from build123d import *

# Parameters (mm, degrees)
SKETCH1_W                                    = 40
SKETCH1_H                                    = 60
BOSS_EXTRUDE1_DEPTH                          = 24
SKETCH4_W                                    = 38
SKETCH4_H                                    = 18
CUT_EXTRUDE2_DEPTH                           = 83
SKETCH5_W                                    = 4
SKETCH5_H                                    = 60
BOSS_EXTRUDE2_DEPTH                          = 5
SKETCH6_W                                    = 4
SKETCH6_H                                    = 11
BOSS_EXTRUDE3_DEPTH                          = 5
SKETCH7_W                                    = 40
SKETCH7_H                                    = 6
BOSS_EXTRUDE4_DEPTH                          = 18
CBORE_FOR_M5_HEXAGON_SOCKET_HEAD_CAP_2_COUNT = 2
CBORE_FOR_M5_HEXAGON_SOCKET_HEAD_CAP_2_PITCH = 24
SKETCH11_W                                   = 4
SKETCH11_H                                   = 5
BOSS_EXTRUDE5_DEPTH                          = 18


with BuildPart() as part:
    # Sketch1 → Boss-Extrude1 (new body)
    with BuildSketch(Plane(origin=(0, 0, 0), x_dir=(1, 0, 0), z_dir=(0, 1, 0))):
        Rectangle(SKETCH1_W, SKETCH1_H)
    extrude(amount=BOSS_EXTRUDE1_DEPTH)

    # Sketch4 → Cut-Extrude2 (cut)
    with BuildSketch(Plane.ZY.offset(20)):
        with Locations((11, 15)):
            Rectangle(SKETCH4_W, SKETCH4_H)
    extrude(amount=-CUT_EXTRUDE2_DEPTH, mode=Mode.SUBTRACT)

    # Sketch5 → Boss-Extrude2 (add)
    with BuildSketch(Plane.XZ):
        Rectangle(SKETCH5_W, SKETCH5_H)
    extrude(amount=BOSS_EXTRUDE2_DEPTH)

    # Sketch6 → Boss-Extrude3 (add)
    with BuildSketch(Plane.XY.offset(30)):
        with Locations((0, 0.5)):
            Rectangle(SKETCH6_W, SKETCH6_H)
    extrude(amount=BOSS_EXTRUDE3_DEPTH)

    # Sketch7 → Boss-Extrude4 (add)
    with BuildSketch(Plane(origin=(0, 6, 0), x_dir=(1, 0, 0), z_dir=(0, 1, 0))):
        with Locations((0, -27)):
            Rectangle(SKETCH7_W, SKETCH7_H)
    extrude(amount=BOSS_EXTRUDE4_DEPTH)

    # Sketch10 → CBORE for M5 Hexagon socket head cap screws1 (revolve, cut)
    with BuildSketch(Plane(origin=(12, 0, -17), x_dir=(0, 0, -1), z_dir=(1, 0, 0))):
        Polygon((0, 0), (0, 24), (2.75, 24), (2.75, 5.7), (5, 5.7), (5, 0.025), (5.025, 0), align=None)
    cbore_for_m5_hexagon_socket_head_cap_scr = revolve(axis=Axis((12, -6.35, -17), (0, 1, 0)), mode=Mode.SUBTRACT)

    # CBORE for M5 Hexagon socket head cap 2: CBORE for M5 Hexagon socket head cap screws1 ×2
    with Locations(*[(-i * CBORE_FOR_M5_HEXAGON_SOCKET_HEAD_CAP_2_PITCH, 0, 0) for i in range(1, CBORE_FOR_M5_HEXAGON_SOCKET_HEAD_CAP_2_COUNT)]):
        add(cbore_for_m5_hexagon_socket_head_cap_scr, mode=Mode.SUBTRACT)

    # Sketch11 → Boss-Extrude5 (add)
    with BuildSketch(Plane(origin=(0, 6, 0), x_dir=(1, 0, 0), z_dir=(0, 1, 0))):
        with Locations((0, -32.5)):
            Rectangle(SKETCH11_W, SKETCH11_H)
    extrude(amount=BOSS_EXTRUDE5_DEPTH)


solid = part.part
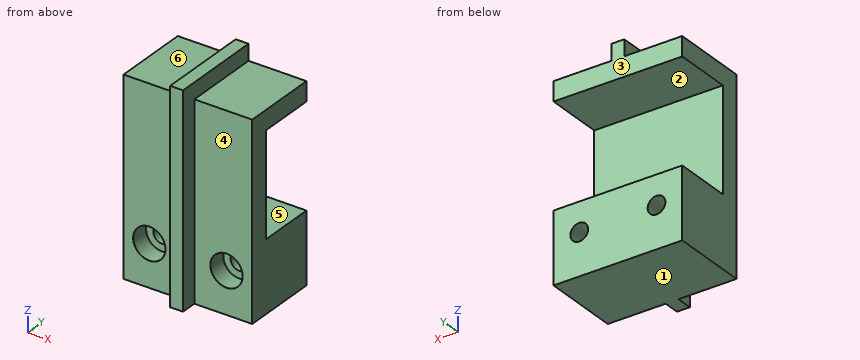
Geometry: final body of the model. Coordinates: model frame, mm. Face numbers are marked on the shaded views. A direction names the side the tool comes from. Give positions to 0.01 mm unless a question says otherwise; leave off trailing zeros. Loops run counter-clockwise (first coordinate to the right, second up) from the corner with the lowest first, then second, coordinate; pieces in that order, holes last. Notation, with made-up numbers: M 75.25,1 L 104.25,1 A18 ccw 104.25,23 Z; hole C 26,-14.5 d4. An arc over 180 degrees is marked long. Put each result on its own line as item: value. Start each with the question number.
1) Contact query for flat-ended pins moving along their axis: pin 1 (8 mm diameter, centred on x = -12.5, z = -19.5, fed in from -Y); pin 2 (1.5 mm diameter, centred on x = 14, y = 21, fed in from +Z); pin 3 (9 mm diameter, centred on x = -12, z = -17, fed in from -Y); pin 4 (3.5 mm diameter, centred on x = 12, z = -17, fed in from +Y). Output: stop coordinate, or through.
2) Pull-direction query (Z, two-part tool) for the marked faces 1, 2 and 3; classes: pulls with the +Z half, pulls with the -Z half, needs draft (parallel to the pull), parting line crosses it, or undercut.
3) Ray query, line 1 along X through (y, z) = (11.5, -17); line 2 along X through (y, z) = (1.2, -17); line 3 along Z through (x, y) = (4.5, 21.5). Return the intervals inside material, ascending.
4) Cut plane B-B (z = -17). Output: boundary loops of the cut face in (x, y) (3 decimals).
5) Cut plane A-A (y = 11.5). Output: boundary loops of the cut face in (x, z), then the cut area to 3 significant figures.
6) Cut plane D-D (z = -23.5). Output: boundary loops of the cut face in (x, y).
7) Cut plane C-C (x = -12). Output: boundary loops of the cut face in (y, z) (3 decimals), then the cut area to 3 significant figures.
8) Access query for the marked faces 4, 5 and 6. Directions: +Z, -Z, +X, -X, +Y, -Y. A direction counts if a zero-diameter tool reaches every point of the face in a straight line with its end or side. Return the directions, or none.
Verdict:
1. pin 1: y = 0
1. pin 2: z = 30
1. pin 3: y = 5.7
1. pin 4: through
2. face 1: pulls with the -Z half
2. face 2: undercut
2. face 3: needs draft
3. line 1: -20 to -14.75, -9.25 to 9.25, 14.75 to 20
3. line 2: -20 to -17, -7 to 7, 17 to 20
3. line 3: -30 to -8, 24 to 30
4. outline: M -20,0 L -17.025,0 L -17,0.025 L -17,5.7 L -14.75,5.7 L -14.75,24 L -20,24 Z; M -9.25,5.7 L -7,5.7 L -7,0.025 L -6.975,0 L -2,0 L -2,-5 L 2,-5 L 2,0 L 6.975,0 L 7,0.025 L 7,5.7 L 9.25,5.7 L 9.25,24 L -9.25,24 Z; M 14.75,5.7 L 17,5.7 L 17,0.025 L 17.025,0 L 20,0 L 20,24 L 14.75,24 Z
5. outline: M -20,-30 L 20,-30 L 20,-8 L -20,-8 Z; M -20,24 L 20,24 L 20,30 L 2,30 L 2,35 L -2,35 L -2,30 L -20,30 Z; hole C -12,-17 d5.5; hole C 12,-17 d5.5
5. area: 1,090 mm2
6. outline: M -20,0 L -2,0 L -2,-5 L 2,-5 L 2,0 L 20,0 L 20,24 L -20,24 Z
7. outline: M 0,-30 L 24,-30 L 24,-19.75 L 5.7,-19.75 L 5.7,-22 L 0.025,-22 L 0,-22.025 Z; M 0,-11.975 L 0.025,-12 L 5.7,-12 L 5.7,-14.25 L 24,-14.25 L 24,-8 L 6,-8 L 6,24 L 24,24 L 24,30 L 0,30 Z
7. area: 706 mm2
8. face 4: +Z, -Z, +X, -Y
8. face 5: +X, -X, +Y
8. face 6: +Z, -X, +Y, -Y
